Verification items for the finished model (mm, model axes). A direction names the side the tool comes from. Coordinates: 2 decimals unless noted, no trailing zeros. Write each loop counter-clockwise with the first axis right and the second up, starting at its lowest first coordinate (ties: lowest second). Pieces come first, ordered by that corner, then holes. Notation, with made-up numbers: M 26,-37 L 77,-37 A8 cw 77,-33 Z; hole C 15.5,-1.5 d6. An arc over 180 degrees is marked long. One line per item, written item: value.
```python
from build123d import *

# Parameters (mm, degrees)
SKETCH1_W           = 60
SKETCH1_H           = 60
BOSS_EXTRUDE1_DEPTH = 10
CUT_EXTRUDE1_DEPTH  = 44.588989435


with BuildPart() as part:
    # Sketch1 → Boss-Extrude1 (new body)
    with BuildSketch(Plane(origin=(0, 0, 0), x_dir=(1, 0, 0), z_dir=(0, 1, 0))):
        Rectangle(SKETCH1_W, SKETCH1_H)
    extrude(amount=BOSS_EXTRUDE1_DEPTH)

    # Sketch2 → Cut-Extrude1 (cut, through all)
    with BuildSketch(Plane(origin=(0, 10, 0), x_dir=(1, 0, 0), z_dir=(0, 1, 0))):
        with BuildLine():
            Line((17.3, 0), (17.3, 20))
            ThreePointArc((17.3, 20), (20, 22.7), (22.7, 20))
            Line((22.7, 20), (22.7, 0))
            ThreePointArc((22.7, 0), (20, -2.7), (17.3, 0))
        make_face()
    cut_extrude1 = extrude(amount=-CUT_EXTRUDE1_DEPTH, mode=Mode.SUBTRACT)

    # Mirror1: Cut-Extrude1 across plane
    add(cut_extrude1.mirror(Plane(origin=(0, 0, 0), x_dir=(0, 0, 1), z_dir=(1, 0, 0))), mode=Mode.SUBTRACT)


solid = part.part
```
Item 1: Cross-section at A-A, the plane z = -5. Enter the section's corners in (x, y), and give its area (3 significant figures).
The answers:
outline: M -30,0 L -22.7,0 L -22.7,10 L -30,10 Z; M -17.3,0 L 17.3,0 L 17.3,10 L -17.3,10 Z; M 22.7,0 L 30,0 L 30,10 L 22.7,10 Z
area: 492 mm²
Item 2: Cross-section at B-B, the plane x = 20. Enter the section's corners in (y, z), and give its area (3 significant figures).
The answers:
outline: M 0,-30 L 10,-30 L 10,-22.7 L 0,-22.7 Z; M 0,2.7 L 10,2.7 L 10,30 L 0,30 Z
area: 346 mm²
Item 3: Cross-section at C-C, the plane y = 8.75. Enter the section's corners in (x, z), and give its area (3 significant figures).
The answers:
outline: M -30,-30 L 30,-30 L 30,30 L -30,30 Z; hole M -22.7,-20 A2.7 ccw -17.3,-20 L -17.3,0 A2.7 ccw -22.7,0 Z; hole M 17.3,-20 A2.7 ccw 22.7,-20 L 22.7,0 A2.7 ccw 17.3,0 Z
area: 3,340 mm²
Item 4: Draft check along Z on faces 3 (the face through (0, 10, 0)), 4 (the face through (0, 5, -30)), 5 (the face through (0, 5, 30)), 6 (the face through (-20.1, 5.1, 2.7)). Enter one of: released by +Z, released by -Z, zero draft, split by the parting line, or undercut.
The answers:
face 3: zero draft
face 4: released by -Z
face 5: released by +Z
face 6: undercut
Item 5: Scan line: line 1 (X direction, y = 3.75, z = -0.5). Record every from-to range of solid material in increasing order.
The answers:
line 1: x = -30 to -22.7, -17.3 to 17.3, 22.7 to 30
Item 6: Access from +Z, -Z, +X, -X, +Y, -Y to the whole of each face (thin tool, end or side, straight path). Record for faces 1 (the face through (-30, 5, 0)), 2 (the face through (-22.7, 5, -10)).
The answers:
face 1: +Z, -Z, -X, +Y, -Y
face 2: +Y, -Y
Item 7: Go/stop test with a flat-tipped pin: P1, Ø6, axis at x = 18.5, z = 2.5, coming from the -Y side. Record where the tip stops, or that it passes through.
The answers:
P1: stops at y = 0
